from build123d import *

# Parameters (mm, degrees)
CUT_EXTRUDE1_DEPTH = 2


with BuildPart() as part:
    # Sketch1 → Revolve1 (revolve)
    with BuildSketch(Plane.XY, mode=Mode.PRIVATE) as revolve1_sk:
        Polygon((-4, 0), (-4, 3.033333333), (-3.533333333, 3.5), (0, 3.5), (0, 2), (19.5699655, 2), (20, 1.5699655), (20, 0), align=None)
    revolve(revolve1_sk.sketch.rotate(Axis((20, 0, 0), (-1, 0, 0)), 270), axis=Axis((20, 0, 0), (-1, 0, 0)))

    # Sketch2 → Cut-Revolve1 (revolve, cut)
    with BuildSketch(Plane.XY, mode=Mode.PRIVATE) as cut_revolve1_sk:
        Polygon((-4, 0), (-4, 1.5), (-2, 1.5), (-1.727022324, 0.75), (20, 0.75), (20, 0), align=None)
    revolve(cut_revolve1_sk.sketch.rotate(Axis((20, 0, 0), (-1, 0, 0)), 270), axis=Axis((20, 0, 0), (-1, 0, 0)), mode=Mode.SUBTRACT)

    # Sketch3 → Cut-Extrude1 (cut)
    with BuildSketch(Plane(origin=(-4, 0, 0), x_dir=(0, 0, -1), z_dir=(1, 0, 0))):
        Polygon((-1.5, 0.866025404), (-1.5, -0.866025404), (0, -1.732050808), (1.5, -0.866025404), (1.5, 0.866025404), (0, 1.732050808), align=None)
    extrude(amount=CUT_EXTRUDE1_DEPTH, mode=Mode.SUBTRACT)


solid = part.part
Could you check a few things on this model? Use its own coordinates, in mm. A direction names the side the tool comes from. Give positions to 0.01 mm unless a question says otherwise; leave off trailing zeros. Order: outer loops, then holes, each group sorted by start corner. A loop starts at its lowest first (then second) coordinate and runs counter-clockwise, first axis right, second up. Notation, with made-up numbers: (-21, 85.5) -> (1, 85.5) arc R17 cw to (1, 106.5) -> close; hole circle Ø9 at (-4, 14.25). An arc over 180 degrees is marked (long way). Return JSON: item names as keys, results as strings.
1. I need wall thicknesses on line 1 (Y direction, x = -0.25, z = 0); line 2 (Y direction, x = 12.25, z = 0); line 3 (X direction, y = 2.75, z = 0.5). Which ranges of each line are inside material? Lowest first, please. Write a range as from..to.
Answer list:
{"line 1": "y = -3.5..-0.75, 0.75..3.5", "line 2": "y = -2..-0.75, 0.75..2", "line 3": "x = -4..0"}
2. For pin 1 Ø1.5 at (x, z) = (2.5, 1) entering from -Y; pin 2 Ø0.6 at (y, z) = (0.5, -1) entering from -X; pin 3 Ø4 at (x, y) = (9.5, -2.5) entering from -Z; pin 4 Ø1 at (x, z) = (15, 3) entering from -Y, each with a flat end and sliding along its axis, tell me the tip position at first contact or that it passes through.
Answer list:
{"pin 1": "stops at y = -1.98", "pin 2": "stops at x = -1.97", "pin 3": "stops at z = -1.94", "pin 4": "passes through"}
3. On a 3-axis mill with a long thin cutter (end or side, diameter ignored), from which of +Z, -Z, +X, -X, +Y, -Y can I reach the whole of each face in a straight line? I mean faces 4 (the flat face through (-3, 0, -1.5)), 5 (the flat face through (20, 0, 1)), 6 (the flat face through (0, -2, 2)). Say none if no direction works.
Answer list:
{"face 4": "-X", "face 5": "+Z, -Z, +X, +Y, -Y", "face 6": "+X"}
4. Imagine slicing it at A-A on x = 15. List the corners of the cut face in (y, z) for me, then the cut area to 3 significant figures.
Answer list:
{"outline": "circle Ø4 at (0, 0); hole circle Ø1.5 at (0, 0)", "area": "10.8 mm2"}
5. Thinking about a two-plate mould opening in Y: for faces 1 (the cylindrical face through (9.289, 0.225, 0.715)), 2 (the cylindrical face through (-1.742, -3.417, -0.759)), 3 (the flat face through (-4, -1.3, -1.3)), which applies, pulls with the +Y half, pulls with the -Y half, needs draft (parallel to the pull), parting line crosses it, or undercut?
Answer list:
{"face 1": "undercut", "face 2": "parting line crosses it", "face 3": "needs draft"}
